from build123d import *

# Parameters (mm, degrees)
SKETCH_2_R                 = 3.96
EXTRUDE_1_DEPTH            = 3.925
EXTRUDE_1_2_DEPTH          = 3.925
EXTRUDE_2_DEPTH            = 1.665
SKETCH_4_R                 = 1.99
EXTRUDE_3_DEPTH            = 2.4975
CHAMFER_1_SIZE             = 0.333
CHAMFER_1_OF_MIRROR_1_SIZE = 0.333


with BuildPart() as part:
    # Sketch 2 → Extrude 1 (new, symmetric)
    with BuildSketch(Plane.XY):
        with Locations((6.35, 0)):
            Circle(SKETCH_2_R)
    extrude(amount=EXTRUDE_1_DEPTH, both=True)



with BuildPart() as body_2:
    # Sketch 2 → Extrude 1 2 (new, symmetric)
    with BuildSketch(Plane.XY):
        with Locations((-6.35, 0)):
            Circle(SKETCH_2_R)
    extrude(amount=EXTRUDE_1_2_DEPTH, both=True)


with BuildPart() as part_1:
    add(part.part)

    add(body_2.part)  # Extrude 2 merges body 2
    # Sketch 3 → Extrude 2 (add)
    with BuildSketch(Plane.XY.offset(3.925)):
        with BuildLine():
            ThreePointArc((-5.213143439, 5.926953869), (-12.385, 0), (-5.213143439, -5.926953869))
            ThreePointArc((-5.213143439, -5.926953869), (0, -5.4315), (5.213143439, -5.926953869))
            ThreePointArc((5.213143439, -5.926953869), (12.385, 0), (5.213143439, 5.926953869))
            ThreePointArc((5.213143439, 5.926953869), (0, 5.4315), (-5.213143439, 5.926953869))
        make_face()
    extrude_2 = extrude(amount=EXTRUDE_2_DEPTH)

    # Sketch 4 → Extrude 3 (add)
    with BuildSketch(Plane.XY.offset(5.59)):
        with Locations((6.35, 0)):
            Circle(SKETCH_4_R)
        with Locations((-6.35, 0)):
            Circle(SKETCH_4_R)
    extrude_3 = extrude(amount=EXTRUDE_3_DEPTH)

    # Chamfer 1
    chamfer_1_edges = [part_1.edges().sort_by_distance(p)[0] for p in [
        (4.36, 0, 8.0875),
        (-8.34, 0, 8.0875),
    ]]
    chamfer(chamfer_1_edges, length=CHAMFER_1_SIZE)

    # Mirror 1: Extrude 2, Extrude 3 across plane
    add(extrude_2.mirror(Plane.XY))
    add(extrude_3.mirror(Plane.XY))

    # Chamfer 1 of Mirror 1
    chamfer_1_of_mirror_1_edges = [part_1.edges().sort_by_distance(p)[0] for p in [
        (4.36, 0, -8.0875),
        (-8.34, 0, -8.0875),
    ]]
    chamfer(chamfer_1_of_mirror_1_edges, length=CHAMFER_1_OF_MIRROR_1_SIZE)


solid = part_1.part
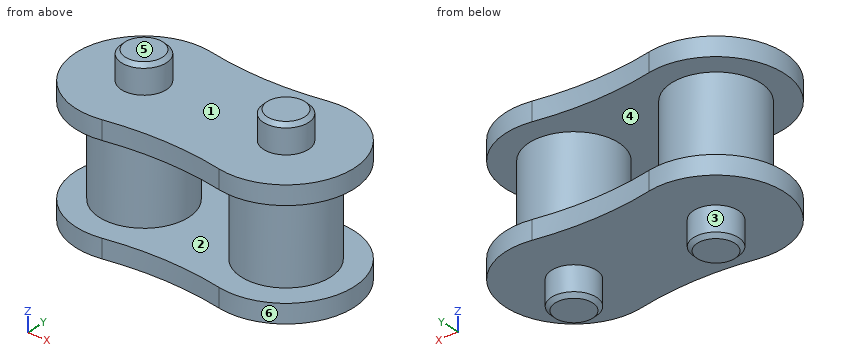
Read the model definition and answer for the solid it produces. Units are mm, in the model's axes. Face numbers are marked on the shaded views. A direction names the side the tool comes from. Round coordinates to 2 decimals unless told otherwise and drop trailing zeros. Write each loop counter-clockwise with the first axis right and the second up, starting at its lowest first coordinate (ties: lowest second). Pieces come first, ordered by that corner, then holes.
Q1. The mould has two halves that part along Z. Classify the marked faces 4, 5 and 6: released by +Z, released by -Z, zero draft, split by the parting line, or undercut.
Values:
face 4: undercut
face 5: released by +Z
face 6: zero draft
Q2. A tool of negligible diameter and unlimited length cuts with its end or side. For the marked faces 1, 2 and 3, from which of +Z, -Z, +X, -X, +Y, -Y can it reach the whole face along a straight path? Write none if from no direction.
Values:
face 1: +Z
face 2: none
face 3: -Z
Q3. Find section C-C on x = 0.5. Determine the outline of the cut face in (y, z) (3 decimals).
Values:
outline: (-5.436, -5.59) - (5.436, -5.59) - (5.436, -3.925) - (-5.436, -3.925) - close; (-5.436, 3.925) - (5.436, 3.925) - (5.436, 5.59) - (-5.436, 5.59) - close
Q4. Find section A-A on x = 6.35. Determine the outline of the cut face in (y, z) (1 decimal).
Values:
outline: (-6, -5.6) - (-2, -5.6) - (-2, -7.8) - (-1.7, -8.1) - (1.7, -8.1) - (2, -7.8) - (2, -5.6) - (6, -5.6) - (6, -3.9) - (4, -3.9) - (4, 3.9) - (6, 3.9) - (6, 5.6) - (2, 5.6) - (2, 7.8) - (1.7, 8.1) - (-1.7, 8.1) - (-2, 7.8) - (-2, 5.6) - (-6, 5.6) - (-6, 3.9) - (-4, 3.9) - (-4, -3.9) - (-6, -3.9) - close
Q5. Straight lines are drawn through the part: line 1 (Z direction, x = -1.75, y = -1.25) (3 decimals); line 2 (Z direction, x = 7.25, y = -2.5); line 3 (X direction, y = -1.5, z = 1.25). For each, find the intervals that lie inside material, in ascending order.
Values:
line 1: z = -5.59 to -3.925, 3.925 to 5.59
line 2: z = -5.59 to 5.59
line 3: x = -10.01 to -2.69, 2.69 to 10.01
Q6. Find section D-D on z = 1. Determine the outline of the cut face in (x, y).
Values:
outline: circle Ø7.92 at (-6.35, 0); circle Ø7.92 at (6.35, 0)
Q7. Find section B-B on z = 6. Determine the outline of the cut face in (x, y).
Values:
outline: circle Ø3.98 at (-6.35, 0); circle Ø3.98 at (6.35, 0)
Q8. Flat-ended cylindrical pins translate along their axes: P1, Ø1, axis at x = 9.5, z = 5.5, coming from the -Y side; P2, Ø1, axis at x = 8.5, y = 3, coming from the -Z side; P3, Ø2, axis at y = 1, z = 2.5, coming from the -X side. Find the tip coordinate at first contact, or state that the pin passes through.
Values:
P1: stops at y = -5.42
P2: stops at z = -5.59
P3: stops at x = -10.31
